For this review, take the finished solid that the model builds, in its own axes (mm). A direction names the side the tool comes from. Give positions to 0.01 mm unless a question says otherwise; leave off trailing zeros. Write each loop counter-clockwise with the first axis right and the second up, starting at its lowest first coordinate (ties: lowest second). Pieces come first, ordered by that corner, then holes.
from build123d import *

# Parameters (mm, degrees)
SKETCH_1_R      = 24
EXTRUDE_1_DEPTH = 5
EXTRUDE_2_DEPTH = 2


with BuildPart() as part:
    # 草图1 → 凸台-拉伸1 (new body)
    with BuildSketch(Plane.XY):
        Circle(SKETCH_1_R)
        with BuildLine():
            Line((-18.33030278, 5), (-14, 5))
            Line((-14, 5), (-14, -5))
            Line((-14, -5), (-18.33030278, -5))
            ThreePointArc((-18.33030278, -5), (0, -19), (18.33030278, -5))
            Line((18.33030278, -5), (14, -5))
            Line((14, -5), (14, 5))
            Line((14, 5), (18.33030278, 5))
            ThreePointArc((18.33030278, 5), (0, 19), (-18.33030278, 5))
        make_face(mode=Mode.SUBTRACT)
    extrude(amount=EXTRUDE_1_DEPTH)

    # 草图2 → 凸台-拉伸2 (add)
    with BuildSketch(Plane.XY.offset(5)):
        with BuildLine():
            Line((-15.822404015, 10.519103156), (-17.943724358, 12.640423499))
            Line((-17.943724358, 12.640423499), (-12.640423499, 17.943724358))
            Line((-12.640423499, 17.943724358), (-10.519103156, 15.822404015))
            ThreePointArc((-10.519103156, 15.822404015), (-13.435028843, 13.435028843), (-15.822404015, 10.519103156))
        make_face()
        with BuildLine():
            Line((10.519103156, 15.822404015), (12.640423499, 17.943724358))
            Line((12.640423499, 17.943724358), (17.943724358, 12.640423499))
            Line((17.943724358, 12.640423499), (15.822404015, 10.519103156))
            ThreePointArc((15.822404015, 10.519103156), (13.435028843, 13.435028843), (10.519103156, 15.822404015))
        make_face()
        with BuildLine():
            Line((15.822404015, -10.519103156), (17.943724358, -12.640423499))
            Line((17.943724358, -12.640423499), (12.640423499, -17.943724358))
            Line((12.640423499, -17.943724358), (10.519103156, -15.822404015))
            ThreePointArc((10.519103156, -15.822404015), (13.435028843, -13.435028843), (15.822404015, -10.519103156))
        make_face()
        with BuildLine():
            Line((-10.519103156, -15.822404015), (-12.640423499, -17.943724358))
            Line((-12.640423499, -17.943724358), (-17.943724358, -12.640423499))
            Line((-17.943724358, -12.640423499), (-15.822404015, -10.519103156))
            ThreePointArc((-15.822404015, -10.519103156), (-13.435028843, -13.435028843), (-10.519103156, -15.822404015))
        make_face()
    extrude(amount=EXTRUDE_2_DEPTH)


solid = part.part
(1) We need section D-D (x = -15). Write out the cut boundary in (y, z) (3 decimals).
(2) We need section A-A (y = 0). Write out the cut boundary in (x, z).
(3) Tool access review of faces 1 (the flat face through (-11.565, -16.868, 5.986)), 2 (the flat face through (16.898, 11.595, 5.986)), 3 (the flat face through (16, -5, 2)), 4 (the flat face through (15.329, -15.255, 5.986)): name each direction out of +Z, -Z, +X, -X, +Y, -Y from which nothing blocks a thin tool from reaching the whole face with its end or side.
(4) We need section B-B (x = 0). Write out the cut boundary in (y, z).
(5) Clearance check with flat-ended pins moving along their axes: pin 1 Ø1.5 at (y, z) = (-1, 2.5) entering from -X; pin 2 Ø3.5 at (x, z) = (16, 2) entering from -Y; pin 3 Ø1.3 at (x, z) = (-15.5, 3) entering from +Y. State where each tip first meets the part, or that it passes through.
(6) The part is to be moulded in two halves that separate along X. For faces 5 (the flat face through (-16, 5, 2)), 6 (the flat face through (15.255, 15.329, 5.986)), 7 (the flat face through (-15.329, 15.255, 5.986)), say which applies: +X half, -X half, draft (parallel to the pull), parting line (faces both ways), or undercut.
(7) We need section C-C (z = 4). Write out the cut boundary in (x, y).
(8) For L1, parallel to Y at x = -0.5, z = 4.5; L2, parallel to Z at x = -4.5, y = -20; L3, parallel to Y at x = 8, z = 4, list the stretches that pass through material, from the lowest coordinate up.
The answers:
1. outline: (-18.735, 0) - (-11.662, 0) - (-11.662, 7) - (-15.584, 7) - (-15.584, 5) - (-18.735, 5) - close; (-5, 0) - (5, 0) - (5, 5) - (-5, 5) - close; (11.662, 0) - (18.735, 0) - (18.735, 5) - (15.584, 5) - (15.584, 7) - (11.662, 7) - close
2. outline: (-24, 0) - (-14, 0) - (-14, 5) - (-24, 5) - close; (14, 0) - (24, 0) - (24, 5) - (14, 5) - close
3. face 1: +Z, -Y
3. face 2: +Z, +X
3. face 3: +Z, -Z
3. face 4: +Z, +X, -Y
4. outline: (-24, 0) - (-19, 0) - (-19, 5) - (-24, 5) - close; (19, 0) - (24, 0) - (24, 5) - (19, 5) - close
5. pin 1: stops at x = -24
5. pin 2: stops at y = -19.31
5. pin 3: stops at y = 18.85
6. face 5: undercut
6. face 6: +X half
6. face 7: -X half
7. outline: circle Ø48 at (0, 0); hole (-18.33, -5) arc R19 ccw to (18.33, -5) - (14, -5) - (14, 5) - (18.33, 5) arc R19 ccw to (-18.33, 5) - (-14, 5) - (-14, -5) - close
8. L1: y = -23.99 to -18.99, 18.99 to 23.99
8. L2: z = 0 to 5
8. L3: y = -22.63 to -17.23, 17.23 to 22.63
